Build history of the part. All positions in model axes, mm. Round coordinates to 2 decimals unless told otherwise and drop trailing zeros. Order: outer loops, then holes, each group sorted by start corner. A loop starts at its lowest first (then second) coordinate and runs counter-clockwise, first axis right, second up. Notation, with made-up numbers: M 2,-27.75 L 21,-27.75 A24 cw 21,-2.75 Z; hole C -4.75,73.5 d4. An arc over 180 degrees is marked long. Use CSV: the item, a comma, the result in double quotes.
from build123d import *

# Parameters (mm, degrees)
SKETCH1_W           = 120
SKETCH1_H           = 120
BOSS_EXTRUDE1_DEPTH = 12
SKETCH2_R           = 56
CUT_EXTRUDE1_DEPTH  = 86.697141143
CIRPATTERN1_COUNT   = 4
CHAMFER1_SIZE       = 2


with BuildPart() as part:
    # Sketch1 → Boss-Extrude1 (new body)
    with BuildSketch(Plane.XY):
        Rectangle(SKETCH1_W, SKETCH1_H)
    extrude(amount=BOSS_EXTRUDE1_DEPTH)

    # Sketch2 → Cut-Extrude1 (cut, through all)
    with BuildSketch(Plane.XY.offset(12)):
        Circle(SKETCH2_R)
    extrude(amount=-CUT_EXTRUDE1_DEPTH, mode=Mode.SUBTRACT)

    # Sketch3 → M8 Clearance Hole1 (revolve, cut)
    with BuildSketch(Plane(origin=(-51.265241636, 51.265241636, 12), x_dir=(0, -1, 0), z_dir=(1, 0, 0))):
        Polygon((0, 0), (0, 52.703872786), (4.5, 50), (4.5, 0), align=None)
    m8_clearance_hole1 = revolve(axis=Axis((-51.265241636, 51.265241636, 18.35), (0, 0, -1)), mode=Mode.SUBTRACT)

    # CirPattern1: M8 Clearance Hole1 ×4 about axis
    cirpattern1_axis = Axis((0, 0, 0), (0, 0, 1))
    for i in range(1, CIRPATTERN1_COUNT):
        add(m8_clearance_hole1.rotate(cirpattern1_axis, i * 360 / CIRPATTERN1_COUNT), mode=Mode.SUBTRACT)

    # Chamfer1
    chamfer1_edges = [part.edges().sort_by_distance(p)[0] for p in [
        (60, -60, 6),
        (-60, -60, 6),
        (-60, 60, 6),
        (60, 60, 6),
    ]]
    chamfer(chamfer1_edges, length=CHAMFER1_SIZE)


solid = part.part
(1) Cut at A-A, the plane x = 0. Give the cut face in (y, z), and give its area (3 significant figures).
Answer block:
outline,"M -60,0 L -56,0 L -56,12 L -60,12 Z; M 56,0 L 60,0 L 60,12 L 56,12 Z"
area,"96.0 mm²"
(2) Cut at C-C, the plane z = 2. Give the cut face in (x, y).
Answer block:
outline,"M -60,-58 L -58,-60 L 58,-60 L 60,-58 L 60,58 L 58,60 L -58,60 L -60,58 Z; hole C 0,0 d112; hole C -51.27,-51.27 d9; hole C -51.27,51.27 d9; hole C 51.27,-51.27 d9; hole C 51.27,51.27 d9"
(3) Wall check: line 1 (Y direction, x = 0, z = 7.75); line 2 (Y direction, x = -49, z = 1.25); line 3 (X direction, y = -48.5, z = 7.25). Give the ranges that are in metal, low to high. Write a range as from..to.
Answer block:
line 1,"y = -60..-56, 56..60"
line 2,"y = -60..-55.15, -47.38..-27.11, 27.11..47.38, 55.15..60"
line 3,"x = -60..-54.82, -47.72..-28, 28..47.72, 54.82..60"
(4) Drop flat-ended pins along their axis: pin 1 (7 mm diameter, centred on x = -51.27, y = 51.27, fed in from -Z); pin 2 (14.5 mm diameter, centred on x = -51.27, y = -51.27, fed in from -Z). Give the stop position or say it passes through.
Answer block:
pin 1,"passes through"
pin 2,"stops at z = 0"
(5) Two-plate mould, pull along Y, no slides. Class faces 1 (the face through (51.73, -21.45, 6.08)), 2 (the face through (-1, 60, 6)), 3 (the face through (60, -1, 6)): released by +Y, released by -Y, zero draft, split by the parting line, or undercut.
Answer block:
face 1,"undercut"
face 2,"released by +Y"
face 3,"zero draft"
